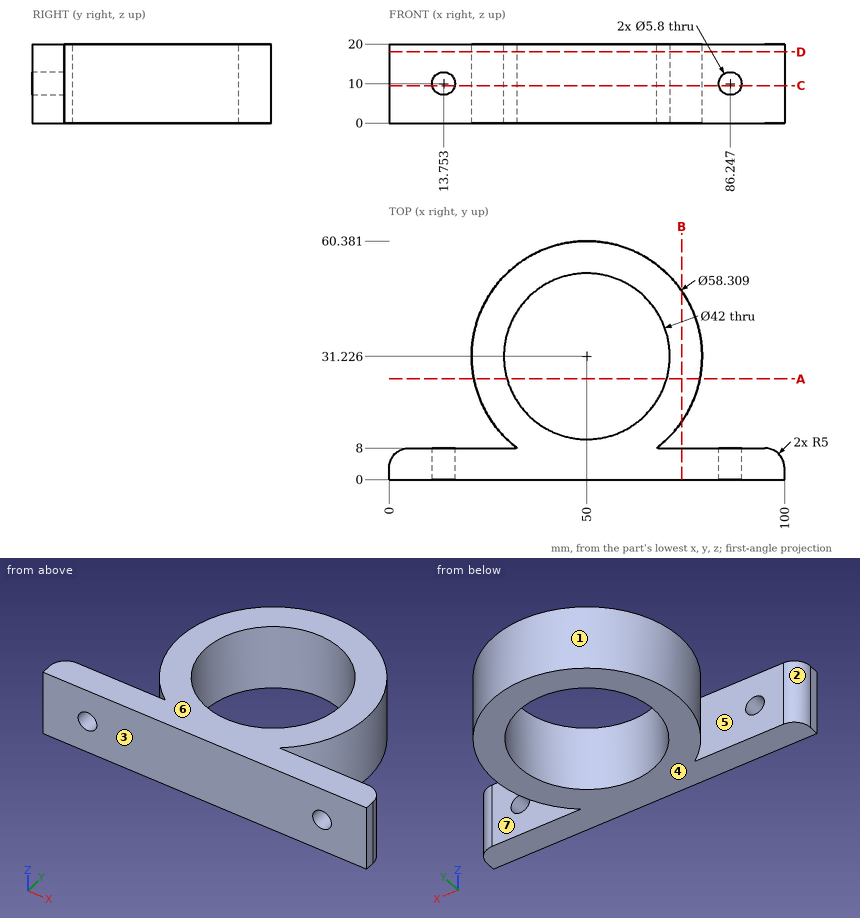
The figure shows three views and two pictorial views of one solid part (mm, origin at its lowest corner). Answer the questions. A direction names the side the tool comes from. Coordinates: 2 decimals unless noted, no trailing zeros. Write each loop counter-clockwise with the first axis right and the second up, starting at its lowest first coordinate (ties: lowest second). Pieces come first, ordered by that corner, then holes.
1. The part is cut by section D-D, the plane z = 18. Write down the section's boundary in (x, y) (1 decimal), and give its area (3 significant figures).
Results list:
outline: (0, 0) - (100, 0) - (100, 3) arc R5 ccw to (95, 8) - (67.6, 8) arc R29.2 ccw (long way) to (32.4, 8) - (5, 8) arc R5 ccw to (0, 3) - close; hole circle Ø42 at (50, 31.2)
area: 1,930 mm2
2. For the marked faces 5, 6 and 7, determine the directions among +Z, -Z, +X, -X, +Y, -Y from which every point of the face is accessible in a straight line to the end or side of a thin tool.
Results list:
face 5: +Z, -Z, -X
face 6: +Z, +X, -X, +Y, -Y
face 7: +Z, -Z, +X
3. For a pull along Y with two mould halves and no side action, classify the marked faces 1, 2, 3 and 4 as +Y half, -Y half, draft (parallel to the pull), parting line (faces both ways), or undercut.
Results list:
face 1: undercut
face 2: +Y half
face 3: -Y half
face 4: draft
4. The part is cut by section B-B, the plane x = 74. Write down the section's boundary in (y, z) (1 decimal), and give its area (3 significant figures).
Results list:
outline: (0, 0) - (8, 0) - (8, 20) - (0, 20) - close; (14.7, 0) - (47.8, 0) - (47.8, 20) - (14.7, 20) - close
area: 822 mm2
5. Consider line 1 along X through (y, z) = (1.5, 10); line 2 along Y through (x, z) = (50, 7); line 3 along X through (y, z) = (3.75, 10). Determine where each line is inside the solid, lowest interval first.
Results list:
line 1: x = 0 to 10.85, 16.65 to 83.35, 89.15 to 100
line 2: y = 0 to 10.23, 52.23 to 60.38
line 3: x = 0.06 to 10.85, 16.65 to 83.35, 89.15 to 99.94
6. The part is cut by section A-A, the plane y = 25.5. Write down the section's boundary in (x, z) (1 decimal), and give its area (3 significant figures).
Results list:
outline: (21.4, 0) - (29.8, 0) - (29.8, 20) - (21.4, 20) - close; (70.2, 0) - (78.6, 0) - (78.6, 20) - (70.2, 20) - close
area: 335 mm2
7. Flat-ended cylindrical pins translate along their axes: pin 1 (12 mm diameter, centred on y = 22, z = 4, fed in from -X) (1 decimal); pin 2 (4 mm diameter, centred on y = 50, z = 4.5, fed in from +X) (1 decimal); pin 3 (4 mm diameter, centred on x = 17.5, z = 15.5, fed in from +Y). Find the tip coordinate at first contact, or state that the pin passes through.
Results list:
pin 1: stops at x = 21
pin 2: stops at x = 73.8
pin 3: stops at y = 8
8. The part is cut by section C-C, the plane z = 9.5. Write down the section's boundary in (x, y) (1 decimal).
Results list:
outline: (0, 0) - (10.9, 0) - (10.9, 8) - (5, 8) arc R5 ccw to (0, 3) - close; (16.6, 0) - (83.4, 0) - (83.4, 8) - (67.6, 8) arc R29.2 ccw (long way) to (32.4, 8) - (16.6, 8) - close; (89.1, 0) - (100, 0) - (100, 3) arc R5 ccw to (95, 8) - (89.1, 8) - close; hole circle Ø42 at (50, 31.2)
